Input: part model. Units: mm. Frame: model coordinates. Face numbers are marked on the shaded views. A direction names the side the tool comes from. Coordinates: 2 decimals unless noted, no trailing zeros. Write each loop counter-clockwise with the first axis right and the second up, starting at its lowest first coordinate (ties: lowest second). Pieces come first, ordered by that corner, then holes. Notation, with made-up numbers: (-2.75, 80) - (14.25, 80) arc R9 ccw to (14.25, 86) - close; hole circle Ø4 at (67, -12.5). An arc over 180 degrees is marked (long way). Put each result on its own line as item: value. Start each with the question number.
1. Cut plane C-C, the plane y = -2.25. Return loops of the section in (x, z).
2. Cut plane D-D, the plane x = -4. Return loops of the section in (y, z).
3. Cut plane A-A, the plane y = 3.25. Return loops of the section in (x, z).
4. Pull-direction query (X, two-part tool) for the marked faces 4, 5 and 6; classes: released by +X, released by -X, zero draft, split by the parting line, or undercut.
5. Pin query (flat end, axial travel): pin 1 (6.5 mm diameter, centred on x = 0, y = 2.5, fed in from +Z); pin 2 (1 mm diameter, centred on x = -2, z = 8, fed in from -Y). Return the tip coordinate at first contact, or that it passes through.
6. Line query: line 1 (Z direction, x = 8.5, y = -5); line 2 (X direction, y = -2, z = 8.75); line 3 (Y direction, x = 0, z = 2). Output: solid intervals per line, ascending.
7. Cut plane B-B, the plane x = 0. Return loops of the section in (y, z).
8. Access query for the marked faces 1, 2 and 3. Directions: +Z, -Z, +X, -X, +Y, -Y. A direction counts if a zero-diameter tool reaches every point of the face in a straight line with its end or side. Return the directions, or none.
from build123d import *

# Parameters (mm, degrees)
SKETCH1_W             = 25
SKETCH1_H             = 20
BOSS_EXTRUDE1_DEPTH   = 10
SKETCH2_W             = 15
SKETCH2_H             = 20
CUT_EXTRUDE1_DEPTH    = 3
M5_TAPPED_HOLE1_D     = 4.2
M5_TAPPED_HOLE2_D     = 4.2
M5_TAPPED_HOLE2_DEPTH = 12.4
M5_TAPPED_HOLE2_TIP   = 1.2618073
CHAMFER1_SIZE         = 0.5


with BuildPart() as part:
    # Sketch1 → Boss-Extrude1 (new body)
    with BuildSketch(Plane.XY):
        Rectangle(SKETCH1_W, SKETCH1_H)
    extrude(amount=BOSS_EXTRUDE1_DEPTH)

    # Sketch2 → Cut-Extrude1 (cut)
    with BuildSketch(Plane.XY.offset(10)):
        Rectangle(SKETCH2_W, SKETCH2_H)
    extrude(amount=-CUT_EXTRUDE1_DEPTH, mode=Mode.SUBTRACT)

    # M5 Tapped Hole1 (through all)
    with Locations(Plane.XY.offset(7)):
        with Locations((0, 2.5)):
            Hole(M5_TAPPED_HOLE1_D / 2)

    # M5 Tapped Hole2
    with Locations(Plane(origin=(0, -10, 0), x_dir=(-1, 0, 0), z_dir=(0, -1, 0))):
        with Locations((8.5, -4), (-8.5, -4)):
            Hole(M5_TAPPED_HOLE2_D / 2, depth=M5_TAPPED_HOLE2_DEPTH)
            with Locations((0, 0, -(M5_TAPPED_HOLE2_DEPTH + M5_TAPPED_HOLE2_TIP / 2))):  # 118° drill point
                Cone(0, M5_TAPPED_HOLE2_D / 2, M5_TAPPED_HOLE2_TIP, mode=Mode.SUBTRACT)

    # Chamfer1
    chamfer1_edges = [part.edges().sort_by_distance(p)[0] for p in [
        (-12.5, 0, 10),
        (-10, -10, 10),
        (-10, 10, 10),
        (10, -10, 10),
        (12.5, 0, 10),
        (0, -10, 0),
        (-12.5, 0, 0),
        (0, 10, 0),
        (12.5, 0, 0),
        (10, 10, 10),
        (12.5, -10, 5),
        (-12.5, -10, 5),
        (-12.5, 10, 5),
        (12.5, 10, 5),
    ]]
    chamfer(chamfer1_edges, length=CHAMFER1_SIZE)


solid = part.part
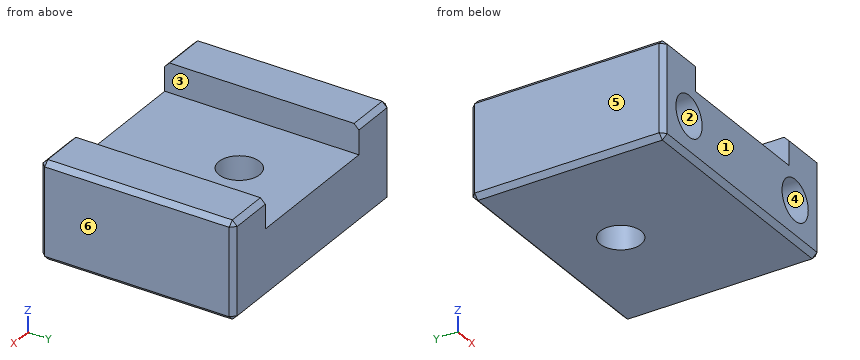
Report:
1. outline: (-12.5, 0.5) - (-12, 0) - (12, 0) - (12.5, 0.5) - (12.5, 9.5) - (12, 10) - (7.5, 10) - (7.5, 7) - (-7.5, 7) - (-7.5, 10) - (-12, 10) - (-12.5, 9.5) - close; hole circle Ø4.2 at (-8.5, 4); hole circle Ø4.2 at (8.5, 4)
2. outline: (-10, 0.5) - (-9.5, 0) - (9.5, 0) - (10, 0.5) - (10, 7) - (-10, 7) - close
3. outline: (-12.5, 0.5) - (-12, 0) - (-1.96, 0) - (-1.96, 7) - (-7.5, 7) - (-7.5, 10) - (-12, 10) - (-12.5, 9.5) - close; (1.96, 0) - (12, 0) - (12.5, 0.5) - (12.5, 9.5) - (12, 10) - (7.5, 10) - (7.5, 7) - (1.96, 7) - close; hole circle Ø1.37 at (-8.5, 4); hole circle Ø1.37 at (8.5, 4)
4. face 4: undercut
4. face 5: released by -X
4. face 6: released by +X
5. pin 1: stops at z = 7
5. pin 2: passes through
6. line 1: z = 0 to 1.9, 6.1 to 10
6. line 2: x = -12.5 to -7.5, 7.5 to 12.5
6. line 3: y = -10 to 0.4, 4.6 to 10
7. outline: (-10, 0.5) - (-9.5, 0) - (0.4, 0) - (0.4, 7) - (-10, 7) - close; (4.6, 0) - (9.5, 0) - (10, 0.5) - (10, 7) - (4.6, 7) - close
8. face 1: +Z, -Z, +X, -X, -Y
8. face 2: -Y
8. face 3: +Z, +Y, -Y
